Study the drawing (mm; zero at the part's minimum x, y, z) and answer. A direction names the side the tool comes from. Round coordinates to 2 decimals unless told otherwise and drop trailing zeros. Loops run counter-clockwise (first coordinate to the right, second up) from the corner with the lowest first, then second, coordinate; pieces in that order, holes last. Notation, with made-up numbers: M 38,46.25 L 56,46.25 A19 cw 56,74.25 Z; hole C 16,65 d3. An arc over 180 degrees is marked long. Write each question's results on one line, items separated by ' | '.
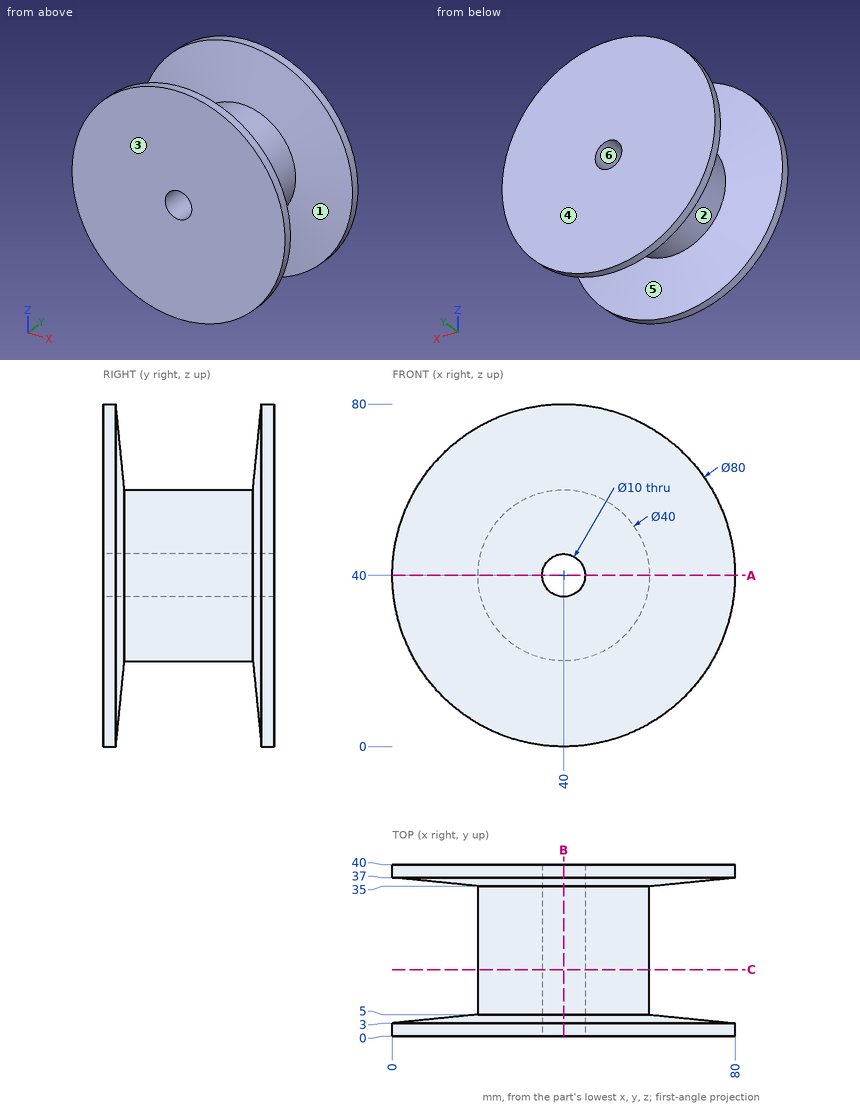
Item 1: The mould has two halves that part along Y. Classify the marked faces 1, 2, 3 and 4: pulls with the +Y half, pulls with the -Y half, needs draft (parallel to the pull), parting line crosses it, or undercut.
Outcome:
face 1: undercut | face 2: undercut | face 3: pulls with the -Y half | face 4: pulls with the +Y half
Item 2: The part is cut by section B-B (x = 40). Determine the outline of the cut face in (y, z).
Outcome:
outline: M 0,0 L 3,0 L 5,20 L 35,20 L 37,0 L 40,0 L 40,35 L 0,35 Z; M 0,45 L 40,45 L 40,80 L 37,80 L 35,60 L 5,60 L 3,80 L 0,80 Z
Item 3: Flat-ended cylindrical pins translate along their axes: pin 1 (3 mm diameter, centred on x = 43.5, y = 10, fed in from +Z); pin 2 (6 mm diameter, centred on y = 25.5, z = 40.5, fed in from +X); pin 3 (6 mm diameter, centred on y = 15, z = 18.5, fed in from -X). Find the tip coordinate at first contact, or state that the pin passes through.
Outcome:
pin 1: stops at z = 59.9 | pin 2: stops at x = 60 | pin 3: stops at x = 32.4
Item 4: For the marked faces 5 and 6, determine the directions among +Z, -Z, +X, -X, +Y, -Y from which every point of the face is accessible in a straight line to the end or side of a thin tool.
Outcome:
face 5: none | face 6: +Y, -Y
Item 5: The part is cut by section C-C (y = 15.5). Determine the outline of the cut face in (x, z), plus the area to 3 significant figures.
Outcome:
outline: C 40,40 d40; hole C 40,40 d10 | area: 1,180 mm2
Item 6: The part is cut by section A-A (z = 40). Determine the outline of the cut face in (x, y), plus the area to 3 significant figures.
Outcome:
outline: M 0,0 L 35,0 L 35,40 L 0,40 L 0,37 L 20,35 L 20,5 L 0,3 Z; M 45,0 L 80,0 L 80,3 L 60,5 L 60,35 L 80,37 L 80,40 L 45,40 Z | area: 1,520 mm2
Item 7: Straight lines are drawn through the part: line 1 (X direction, y = 23, z = 40); line 2 (Z direction, x = 44, y = 23). For each, find the intervals that lie inside material, in ascending order.
Outcome:
line 1: x = 20 to 35, 45 to 60 | line 2: z = 20.4 to 37, 43 to 59.6
